Build history of the part. All positions in model axes, mm. A direction names the side the tool comes from. Round coordinates to 2 decimals unless told otherwise and drop trailing zeros. Loops run counter-clockwise (first coordinate to the right, second up) from the corner with the lowest first, then second, coordinate; pieces in that order, holes last. Notation, with made-up numbers: (3.5, 61) -> (24.5, 61) arc R20 cw to (24.5, 77) -> close; hole circle Ø2 at (-2, -22). An arc over 180 degrees is marked (long way). Put each result on its own line as item: value. Start each with the question number.
```python
from build123d import *

# Parameters (mm, degrees)
CROSS_FLANGE_DEPTH        = 5
SKETCH1_3_R               = 5
SHAFT_150_DEPTH           = 150
ARM_HOLES_A_SKETCH_R      = 1.5
ARM_HOLES_A_DEPTH         = 158.863865403
ARM_HOLES_B_SKETCH_R      = 1.5
ARM_HOLES_B_DEPTH         = 158.863865403
CENTER_RECESS_10_SKETCH_R = 5
CENTER_RECESS_10_X2_DEPTH = 2


with BuildPart() as part:
    # Cross Flange Profile → Cross Flange (new, symmetric)
    with BuildSketch(Plane.XY):
        with BuildLine():
            Line((-4, 14.456832295), (-4, 30))
            Line((-4, 30), (-9, 30))
            Line((-9, 30), (-9, 12))
            ThreePointArc((-9, 12), (-10.606601718, 10.606601718), (-12, 9))
            Line((-12, 9), (-30, 9))
            Line((-30, 9), (-30, 4))
            Line((-30, 4), (-14.456832295, 4))
            ThreePointArc((-14.456832295, 4), (-15, 0), (-14.456832295, -4))
            Line((-14.456832295, -4), (-30, -4))
            Line((-30, -4), (-30, -9))
            Line((-30, -9), (-12, -9))
            ThreePointArc((-12, -9), (-10.606601718, -10.606601718), (-9, -12))
            Line((-9, -12), (-9, -30))
            Line((-9, -30), (-4, -30))
            Line((-4, -30), (-4, -14.456832295))
            ThreePointArc((-4, -14.456832295), (0, -15), (4, -14.456832295))
            Line((4, -14.456832295), (4, -30))
            Line((4, -30), (9, -30))
            Line((9, -30), (9, -12))
            ThreePointArc((9, -12), (10.606601718, -10.606601718), (12, -9))
            Line((12, -9), (30, -9))
            Line((30, -9), (30, -4))
            Line((30, -4), (14.456832295, -4))
            ThreePointArc((14.456832295, -4), (15, 0), (14.456832295, 4))
            Line((14.456832295, 4), (30, 4))
            Line((30, 4), (30, 9))
            Line((30, 9), (12, 9))
            ThreePointArc((12, 9), (10.606601718, 10.606601718), (9, 12))
            Line((9, 12), (9, 30))
            Line((9, 30), (4, 30))
            Line((4, 30), (4, 14.456832295))
            ThreePointArc((4, 14.456832295), (0, 15), (-4, 14.456832295))
        make_face()
    extrude(amount=CROSS_FLANGE_DEPTH, both=True)

    # Sketch1_3 → Shaft 150 (add)
    with BuildSketch(Plane.XY):
        Circle(SKETCH1_3_R)
    extrude(amount=-SHAFT_150_DEPTH)

    # Arm Holes A Sketch → Arm Holes A (cut, through all)
    with BuildSketch(Plane(origin=(9, 0, 0), x_dir=(0, 0, -1), z_dir=(1, 0, 0))):
        with BuildLine():
            ThreePointArc((0, -30), (-3.535533906, -28.535533906), (-5, -25))
            Line((-5, -25), (-5, -30))
            Line((-5, -30), (0, -30))
        make_face()
        with BuildLine():
            ThreePointArc((5, -25), (3.535533906, -28.535533906), (0, -30))
            Line((0, -30), (5, -30))
            Line((5, -30), (5, -25))
        make_face()
        with BuildLine():
            Line((-5, 30), (-5, 25))
            ThreePointArc((-5, 25), (-3.535533906, 28.535533906), (0, 30))
            Line((0, 30), (-5, 30))
        make_face()
        with BuildLine():
            Line((5, 30), (0, 30))
            ThreePointArc((0, 30), (3.535533906, 28.535533906), (5, 25))
            Line((5, 25), (5, 30))
        make_face()
        with Locations(Location((0, 25, 0), (0, 0, 90))):
            Circle(ARM_HOLES_A_SKETCH_R)
        with Locations(Location((0, -25, 0), (0, 0, 90))):
            Circle(ARM_HOLES_A_SKETCH_R)
    extrude(amount=-ARM_HOLES_A_DEPTH, mode=Mode.SUBTRACT)

    # Arm Holes B Sketch → Arm Holes B (cut, through all)
    with BuildSketch(Plane(origin=(0, 9, 0), x_dir=(1, 0, 0), z_dir=(0, 1, 0))):
        with BuildLine():
            ThreePointArc((30, 0), (28.535533906, -3.535533906), (25, -5))
            Line((25, -5), (30, -5))
            Line((30, -5), (30, 0))
        make_face()
        with BuildLine():
            ThreePointArc((25, 5), (28.535533906, 3.535533906), (30, 0))
            Line((30, 0), (30, 5))
            Line((30, 5), (25, 5))
        make_face()
        with BuildLine():
            Line((-30, -5), (-25, -5))
            ThreePointArc((-25, -5), (-28.535533906, -3.535533906), (-30, 0))
            Line((-30, 0), (-30, -5))
        make_face()
        with BuildLine():
            Line((-30, 5), (-30, 0))
            ThreePointArc((-30, 0), (-28.535533906, 3.535533906), (-25, 5))
            Line((-25, 5), (-30, 5))
        make_face()
        with Locations(Location((-25, 0, 0), (0, 0, 180))):
            Circle(ARM_HOLES_B_SKETCH_R)
        with Locations((25, 0)):
            Circle(ARM_HOLES_B_SKETCH_R)
    extrude(amount=-ARM_HOLES_B_DEPTH, mode=Mode.SUBTRACT)

    # Center Recess _10 Sketch → Center Recess _10 x2 (cut)
    with BuildSketch(Plane.XY.offset(5)):
        Circle(CENTER_RECESS_10_SKETCH_R)
    extrude(amount=-CENTER_RECESS_10_X2_DEPTH, mode=Mode.SUBTRACT)


solid = part.part
```
Item 1: Cut at A-A on y = 18. Write the cut outline in (x, z), then the cut area to 3 significant figures.
Item 2: Cut at D-D on z = -30. Write the cut outline in (x, y), then the cut area to 3 significant figures.
Item 3: Cut at B-B on x = -7.5. Write the cut outline in (y, z), then the cut area to 3 significant figures.
Item 4: Pull direction Y, two halves, no side cores. Call faces 5 (the face through (10.628, 10.586, 0.07)), 6 (the face through (15, 0, 0)), 7 (the face through (0, 6, -5)): +Y half, -Y half, draft (parallel to the pull), parting line (faces both ways), or undercut.
Item 5: Drop flat-ended pins along their axis: pin 1 (11 mm diameter, centred on x = 23.5, z = -2, fed in from +Y); pin 2 (3 mm diameter, centred on y = 25, z = 1.5, fed in from +X); pin 3 (11 mm diameter, centred on x = 22.5, z = 0.5, fed in from -Y); pin 4 (11 mm diameter, centred on x = -1, y = 1.5, fed in from +Z). Give the stop position or say it passes through.
Item 6: 3-axis set-ups, long thin cutter, end or side, ignore diameter. For faces 1 (the face through (9, -21, 0)), 2 (the face through (-22, 4, 0)), 3 (the face through (4, 22, 0)), 4 (the face through (-1.08, -4.88, 4.01)): which of +Z, -Z, +X, -X, +Y, -Y reach the whole face in a straight line?
Item 7: Wall check: line 1 (Z direction, x = 5, y = 25); line 2 (Z direction, x = 5, y = 12); line 3 (X direction, y = 3, z = -13). Give the ranges that are in metal, low to high. Write a range as from..to.
Item 8: Cut at C-C on y = 0. Write the cut outline in (x, z), then the cut area to 3 significant figures.
Ans:
1. outline: (-9, -5) -> (-4, -5) -> (-4, 5) -> (-9, 5) -> close; (4, -5) -> (9, -5) -> (9, 5) -> (4, 5) -> close
1. area: 100 mm2
2. outline: circle Ø10 at (0, 0)
2. area: 78.5 mm2
3. outline: (-25, -5) -> (25, -5) arc R5 ccw to (25, 5) -> (-25, 5) arc R5 ccw to start; hole circle Ø3 at (-25, 0); hole circle Ø3 at (25, 0)
3. area: 564 mm2
4. face 5: +Y half
4. face 6: undercut
4. face 7: draft
5. pin 1: stops at y = 9
5. pin 2: stops at x = 9
5. pin 3: stops at y = -9
5. pin 4: stops at z = 5
6. face 1: +Z, -Z, +X, -Y
6. face 2: +Z, -Z, -X
6. face 3: +Z, -Z, +Y
6. face 4: +Z
7. line 1: z = -5..-1.5, 1.5..5
7. line 2: z = -5..5
7. line 3: x = -4..4
8. outline: (-15, -5) -> (-5, -5) -> (-5, -150) -> (5, -150) -> (5, -5) -> (15, -5) -> (15, 5) -> (5, 5) -> (5, 3) -> (-5, 3) -> (-5, 5) -> (-15, 5) -> close
8. area: 1,730 mm2
